Verification items for this drawing (mm, ordinates from the low corner). Give positions to 0.01 mm unless a question says otherwise; leave off trailing zeros. Loops run counter-clockwise (first coordinate to the right, second up) from the corner with the lowest first, then second, coordinate; pieces in that order, holes last. Notation, with made-up numbers: M 89.5,26 L 115.5,26 A15 ccw 115.5,53 Z; hole C 28,-34.75 d10. An arc over 180 degrees is marked long. Answer in a Markdown table with one row per item.
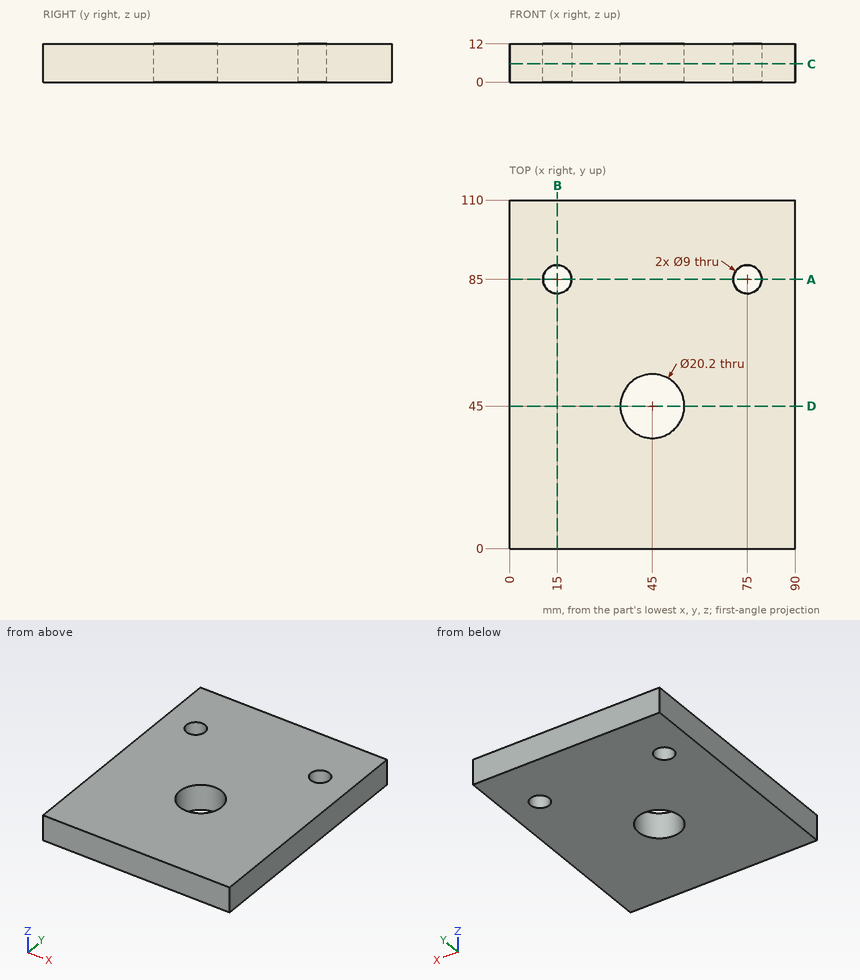
Item 1: Scan lines: L1, parallel to X at y = 85, z = 8; L2, parallel to Y at x = 45, z = 6; L3, parallel to Y at x = 75, z = 7. Record each from-to range of solid material in increasing order. Write a range as [from, to].
Reported:
| item | result |
|---|---|
| L1 | x = [0, 10.5], [19.5, 70.5], [79.5, 90] |
| L2 | y = [0, 34.9], [55.1, 110] |
| L3 | y = [0, 80.5], [89.5, 110] |
Item 2: Go/stop test with a flat-tipped pin: pin 1 (8 mm diameter, centred on x = 75, y = 85, fed in from +Z). Record where the tip stops, or that it passes through.
Reported:
| item | result |
|---|---|
| pin 1 | passes through |
Item 3: Sectioned sample at D-D (y = 45). Record the cut outline in (x, z), and give its area (3 significant figures).
Reported:
| item | result |
|---|---|
| outline | M 0,0 L 34.9,0 L 34.9,12 L 0,12 Z; M 55.1,0 L 90,0 L 90,12 L 55.1,12 Z |
| area | 838 mm^2 |
Item 4: Sectioned sample at C-C (z = 5.75). Record the cut outline in (x, y), and give its area (3 significant figures).
Reported:
| item | result |
|---|---|
| outline | M 0,0 L 90,0 L 90,110 L 0,110 Z; hole C 15,85 d9; hole C 45,45 d20.2; hole C 75,85 d9 |
| area | 9,450 mm^2 |
Item 5: Sectioned sample at B-B (x = 15). Record the cut outline in (y, z), and give its area (3 significant figures).
Reported:
| item | result |
|---|---|
| outline | M 0,0 L 80.5,0 L 80.5,12 L 0,12 Z; M 89.5,0 L 110,0 L 110,12 L 89.5,12 Z |
| area | 1,210 mm^2 |
Item 6: Sectioned sample at A-A (y = 85). Record the cut outline in (x, z), and give its area (3 significant figures).
Reported:
| item | result |
|---|---|
| outline | M 0,0 L 10.5,0 L 10.5,12 L 0,12 Z; M 19.5,0 L 70.5,0 L 70.5,12 L 19.5,12 Z; M 79.5,0 L 90,0 L 90,12 L 79.5,12 Z |
| area | 864 mm^2 |
